Verification items for this drawing (mm, ordinates from the low corner). A direction names the side the tool comes from. Round coordinates to 2 decimals unless told otherwise and drop trailing zeros. Order: outer loops, then holes, each group sorted by start corner. A loop starts at its lowest first (then second) coordinate and runs counter-clockwise, first axis right, second up. Notation, with made-up numbers: (-19, 1.5) -> (2, 1.5) arc R4 cw to (2, 8.5) -> close; hole circle Ø9 at (26.5, 61.5). An arc over 180 degrees is marked (long way). Return JSON: item names as keys, results as strings. Group by question number.
Item 1: Access from +Z, -Z, +X, -X, +Y, -Y to the whole of each face (thin tool, end or side, straight path). Record for the marked faces 1, 2 and 3.
Item 2: Scan lines: probe 1 along Y at (x, z) = (15, 3); probe 2 along Y at (x, z) = (7, 9); probe 3 along Z at (x, y) = (7.75, 25). Record each from-to range of solid material in increasing order. Write a range as from..to.
Item 3: Depth check by flat-ended pin: pin 1 Ø1.5 at (y, z) = (25.5, 14.5) entering from -X; pin 2 Ø2 at (x, y) = (15, 18.5) entering from -Z; pin 3 Ø4 at (x, y) = (13, 38.5) entering from -Z. Enter the tip coordinate at first touch or a pass-through.
Item 4: Sectioned sample at B-B on x = 10. Record the cut outline in (y, z), plus the area to 3 significant figures.
Item 5: Sectioned sample at A-A on z = 10. Record the cut outline in (x, y), plus the area to 3 significant figures.
Item 6: Sectioned sample at C-C on y = 13.5. Record the cut outline in (x, z).
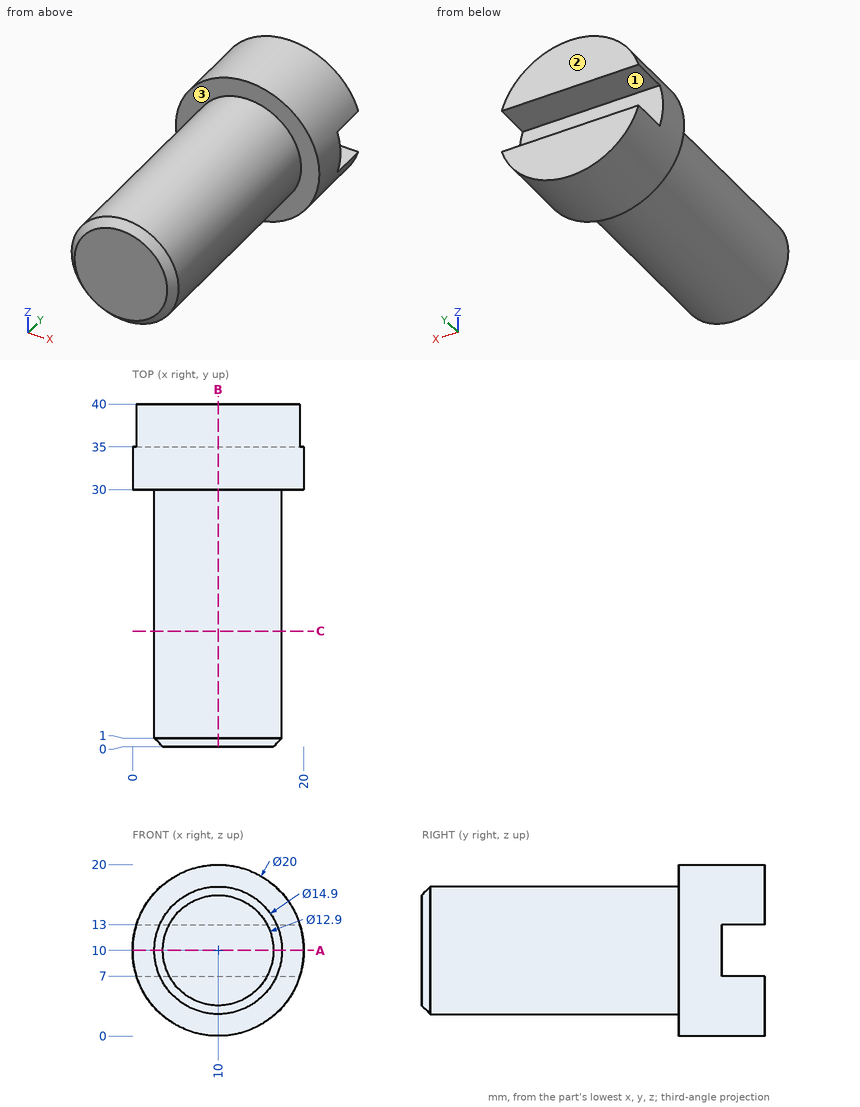
Recorded:
{
 "1": {"face 1": "+X, -X, +Y", "face 2": "+Z, -Z, +X, -X, +Y", "face 3": "-Y"},
 "2": {"probe 1": "30..40", "probe 2": "0..35", "probe 3": "2.9..17.1"},
 "3": {"pin 1": "x = 3.56", "pin 2": "z = 3.71", "pin 3": "z = 0.05"},
 "4": {"outline": "(0, 3.55) -> (1, 2.55) -> (30, 2.55) -> (30, 0) -> (40, 0) -> (40, 7) -> (35, 7) -> (35, 13) -> (40, 13) -> (40, 20) -> (30, 20) -> (30, 17.45) -> (1, 17.45) -> (0, 16.45) -> close", "area": "616 mm²"},
 "5": {"outline": "(0, 30) -> (2.55, 30) -> (2.55, 1) -> (3.55, 0) -> (16.45, 0) -> (17.45, 1) -> (17.45, 30) -> (20, 30) -> (20, 35) -> (0, 35) -> close", "area": "546 mm²"},
 "6": {"outline": "circle Ø14.9 at (10, 10)"}
}
